Verification items for this drawing (mm, ordinates from the low corner). Round coordinates to 2 decimals unless told otherwise and drop trailing zeros. Order: outer loops, then holes, each group sorted by start corner. A loop starts at its lowest first (then second) coordinate and runs counter-clockwise, first axis right, second up. Notation, with made-up numbers: (64.5, 47.25) - (105.5, 47.25) arc R9 ccw to (105.5, 58.25) - close; hole circle Ø2 at (29.5, -13.5). An arc over 180 degrees is marked (long way). Return JSON: item names as keys, results as strings. Group by question number.
Q1. Material ranges on line 1 along Y through (x, z) = (21.5, 53.5); line 2 along X through (y, z) = (4.5, 3); line 3 along Y through (x, z) = (1.5, 37.5), recorded low to high.
Q2. Gauge pin test, flat ends, axial feed: pin 1 Ø3 at (y, z) = (15, 46) entering from +X; pin 2 Ø1.5 at (x, z) = (10, 37.5) entering from -Y; pin 3 Ø4 at (y, z) = (7, 40) entering from -X. Record the tip position at first contact, or that the pin passes through.
Q3. Sectioned sample at A-A, the plane z = 17. Record the cut outline in (x, y), then the cut area to 3 significant figures.
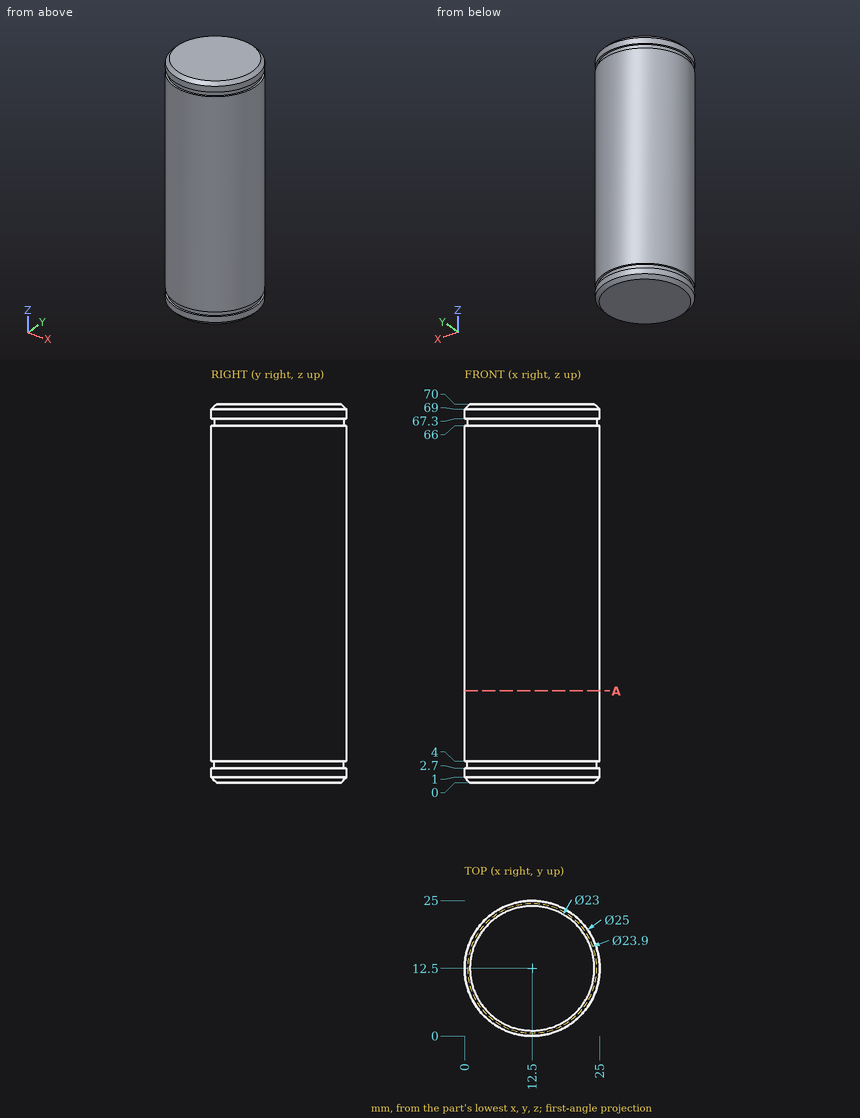
Reply:
{
 "1": {"line 1": "3.83 to 21.17", "line 2": "3.62 to 21.38", "line 3": "6.56 to 18.44"},
 "2": {"pin 1": "x = 24.96", "pin 2": "y = 0.12", "pin 3": "x = 0.5"},
 "3": {"outline": "circle Ø25 at (12.5, 12.5)", "area": "491 mm^2"}
}
